Build history of the part. All positions in model axes, mm. A direction names the side the tool comes from. Round coordinates to 2 decimals unless told otherwise and drop trailing zeros. Write each loop counter-clockwise with the first axis right and the second up, starting at its lowest first coordinate (ties: lowest second). Pieces come first, ordered by that corner, then holes. Notation, with made-up numbers: (-21, -24) -> (-17, -24) arc R21 ccw to (-17, 7) -> close; hole circle Ø1 at (87, -38). An arc over 180 degrees is marked (long way). Return JSON: item names as keys, results as strings.
from build123d import *

# Parameters (mm, degrees)
SKETCH2_R = 5.08


with BuildPart() as part:
    # Sweep1: sweep along a path in Sketch1
    with BuildLine(Plane(origin=(0, 0, 0), x_dir=(0, 0, -1), z_dir=(1, 0, 0))) as sweep1_path:
        Line((-76.2, 57.15), (-76.2, 88.9))
        ThreePointArc((-76.2, 88.9), (-72.480256121, 97.880256121), (-63.5, 101.6))
        Line((-63.5, 101.6), (63.5, 101.6))
        ThreePointArc((63.5, 101.6), (72.480256121, 97.880256121), (76.2, 88.9))
        Line((76.2, 88.9), (76.2, 57.15))
    # Sketch2 → Sweep1 (sweep)
    with BuildSketch(Plane(origin=(0, 57.15, 76.2), x_dir=(-1, 0, 0), z_dir=(0, 1, 0))):
        Circle(SKETCH2_R)
    sweep(path=sweep1_path.line)


solid = part.part
Q1. Saw through at A-A on x = 0. List the corners of the cut face in (y, z), then the cut area to 3 significant figures.
Verdict:
{"outline": "(57.15, -81.28) -> (88.9, -81.28) arc R17.78 ccw to (106.68, -63.5) -> (106.68, 63.5) arc R17.78 ccw to (88.9, 81.28) -> (57.15, 81.28) -> (57.15, 71.12) -> (88.9, 71.12) arc R7.62 cw to (96.52, 63.5) -> (96.52, -63.5) arc R7.62 cw to (88.9, -71.12) -> (57.15, -71.12) -> close", "area": "2,340 mm²"}
Q2. 3-axis set-ups, long thin cutter, end or side, ignore diameter. For faces 1 (the cylindrical face through (0.661, 72.803, -81.237)), 2 (the flat face through (0, 57.15, -76)): which of +Z, -Z, +X, -X, +Y, -Y reach the whole face in a straight line?
Verdict:
{"face 1": "-Y", "face 2": "+Z, -Z, +X, -X, -Y"}
Q3. Wall check: L1, parallel to Z at x = 0.5, y = 77.5; L2, parallel to Z at x = 2.25, y = 86; L3, parallel to Y at x = 0, z = 29.5. Give the ranges that are in metal, low to high.
Verdict:
{"L1": "z = -81.26 to -71.14, 71.14 to 81.26", "L2": "z = -80.75 to -71.65, 71.65 to 80.75", "L3": "y = 96.52 to 106.68"}
Q4. Saw through at B-B on y = 69.5. List the corners of the cut face in (x, z), then the cut area to 3 significant figures.
Verdict:
{"outline": "circle Ø10.16 at (0, -76.2); circle Ø10.16 at (0, 76.2)", "area": "162 mm²"}
Q5. Two-plate mould, pull along Z, no slides. Class faces 3 (the cylindrical face through (1.1, 96.64, -0.89)), 4 (the flat face through (0, 57.15, 76)): +Z half, -Z half, draft (parallel to the pull), parting line (faces both ways), or undercut.
Verdict:
{"face 3": "undercut", "face 4": "draft"}
Q6. Saw through at C-C on z = -59. List the corners of the cut face in (x, y), then the cut area to 3 significant figures.
Verdict:
{"outline": "circle Ø10.16 at (0, 101.6)", "area": "81.1 mm²"}
Q7. Pin check, flat tips, straight feed: pin 1 Ø4 at (x, y) = (4, 87) entering from +Z; pin 2 Ø2 at (x, y) = (-3, 98) entering from +Z; pin 3 Ø1.5 at (x, y) = (3.5, 90.5) entering from -Z. Stop position of each tip, or through.
Verdict:
{"pin 1": "stops at z = 80.87", "pin 2": "stops at z = 78.55", "pin 3": "stops at z = -80.4"}
